from build123d import *

# Parameters (mm, degrees)
CHAMFER1_SIZE  = 3
CHAMFER1_SIZE2 = 0.803847577


with BuildPart() as part:
    # Sketch1 → Revolve1 (revolve)
    with BuildSketch(Plane.XY, mode=Mode.PRIVATE) as revolve1_sk:
        Polygon((26, 31), (42.5, 31), (42.5, 3), (54, 3), (54, 0), (57.5, 0), (57.5, -8), (26, -8), align=None)
    revolve(revolve1_sk.sketch.rotate(Axis((0, 0, 0), (0, 1, 0)), 90), axis=Axis((0, 0, 0), (0, 1, 0)))

    # Chamfer1
    chamfer1_edges = [part.edges().sort_by_distance(p)[0] for p in [
        (0, 31, 42.5),
    ]]
    chamfer1_side = [part.faces().sort_by_distance(p)[0] for p in [
        (0, 17, 42.5),
    ]]
    chamfer(chamfer1_edges, length=CHAMFER1_SIZE, length2=CHAMFER1_SIZE2, reference=chamfer1_side[0])


solid = part.part
Verification items for the finished model (mm, model axes). A direction names the side the tool comes from. Coordinates: 2 decimals unless noted, no trailing zeros. Loops run counter-clockwise (first coordinate to the right, second up) from the corner with the lowest first, then second, coordinate; pieces in that order, holes last. Notation, with made-up numbers: (35.25, -36.75) -> (79.25, -36.75) arc R17 ccw to (79.25, -14.75) -> close; hole circle Ø6 at (47, 70). An arc over 180 degrees is marked (long way). Answer as a JSON object with one key per item and string values. Group by question number.
Item 1: Sectioned sample at B-B on z = 0. Record the boundary of the cut face in (x, y), plus the area to 3 significant figures.
Item 2: Sectioned sample at C-C on y = -2. Record the boundary of the cut face in (x, z), plus the area to 3 significant figures.
Item 3: Depth check by flat-ended pin: pin 1 (1 mm diameter, centred on y = 4.5, z = -15, fed in from -X); pin 2 (6 mm diameter, centred on x = -14, y = 15, fed in from +Z); pin 3 (3 mm diameter, centred on y = 24, z = 22.5, fed in from +X). Enter the tip coordinate at first touch or a pass-through.
Item 4: Sectioned sample at A-A on x = 0. Record the boundary of the cut face in (y, z).
Item 5: Mould release check, pull along X, two halves, no side actions. Record for faces 1 (the cylindrical face through (15.821, 11.773, 20.633)), 2 (the cylindrical face through (56.133, -4.056, 12.465)), 3 (the flat face through (12, -8, -25)): +X half, -X half, draft (parallel to the pull), parting line (faces both ways), or undercut.
Item 6: Tool access check on faces 4 (the flat face through (-19, 31, 18)), 5 (the cylindrical face through (-12.766, 15.325, -40.537)). Record the directions out of +Z, -Z, +X, -X, +Y, -Y that give a thin tool (end or side, any length) a straight path to the whole face; none if there is none.
Item 7: Scan lines: probe 1 along X at (y, z) = (15, 0); probe 2 along X at (y, z) = (1, 0); probe 3 along Y at (x, z) = (-47, -31.5). Record each from-to range of solid material in increasing order.
Item 8: Sectioned sample at D-D on z = 44. Record the boundary of the cut face in (x, y).
Evaluation:
{
 "1": {"outline": "(-57.5, -8) -> (-26, -8) -> (-26, 31) -> (-41.7, 31) -> (-42.5, 28) -> (-42.5, 3) -> (-54, 3) -> (-54, 0) -> (-57.5, 0) -> close; (26, -8) -> (57.5, -8) -> (57.5, 0) -> (54, 0) -> (54, 3) -> (42.5, 3) -> (42.5, 28) -> (41.7, 31) -> (26, 31) -> close", "area": "1,590 mm²"},
 "2": {"outline": "circle Ø115 at (0, 0); hole circle Ø52 at (0, 0)", "area": "8,260 mm²"},
 "3": {"pin 1": "stops at x = -39.95", "pin 2": "stops at z = 41.05", "pin 3": "stops at x = 36.95"},
 "4": {"outline": "(-8, -57.5) -> (0, -57.5) -> (0, -54) -> (3, -54) -> (3, -42.5) -> (28, -42.5) -> (31, -41.7) -> (31, -26) -> (-8, -26) -> close; (-8, 26) -> (31, 26) -> (31, 41.7) -> (28, 42.5) -> (3, 42.5) -> (3, 54) -> (0, 54) -> (0, 57.5) -> (-8, 57.5) -> close"},
 "5": {"face 1": "undercut", "face 2": "parting line", "face 3": "draft"},
 "6": {"face 4": "+Z, -Z, +X, -X, +Y", "face 5": "+Y"},
 "7": {"probe 1": "x = -42.5 to -26, 26 to 42.5", "probe 2": "x = -54 to -26, 26 to 54", "probe 3": "y = -8 to 0"},
 "8": {"outline": "(-37.02, -8) -> (37.02, -8) -> (37.02, 0) -> (31.3, 0) -> (31.3, 3) -> (-31.3, 3) -> (-31.3, 0) -> (-37.02, 0) -> close"}
}
